```python
from build123d import *

# Parameters (mm, degrees)
SKETCH1_W              = 200
SKETCH1_H              = 60
BOSS_EXTRUDE1_DEPTH    = 12
M12_TAPPED_HOLE1_D     = 10.2
M12_TAPPED_HOLE1_DEPTH = 29.25
M12_TAPPED_HOLE1_TIP   = 3.064389157


with BuildPart() as part:
    # Sketch1 → Boss-Extrude1 (new body)
    with BuildSketch(Plane.XY):
        Rectangle(SKETCH1_W, SKETCH1_H)
    extrude(amount=BOSS_EXTRUDE1_DEPTH)

    # M12 Tapped Hole1
    with Locations(Plane.XY.offset(12)):
        with Locations((-80, 5), (80, 5)):
            Hole(M12_TAPPED_HOLE1_D / 2, depth=M12_TAPPED_HOLE1_DEPTH)
            with Locations((0, 0, -(M12_TAPPED_HOLE1_DEPTH + M12_TAPPED_HOLE1_TIP / 2))):  # 118° drill point
                Cone(0, M12_TAPPED_HOLE1_D / 2, M12_TAPPED_HOLE1_TIP, mode=Mode.SUBTRACT)


solid = part.part
```
Check sheet for the modelled part. Datum: model origin and axes. Units: mm. Give positions to 0.01 mm unless a question says otherwise; leave off trailing zeros. Write each loop counter-clockwise with the first axis right and the second up, starting at its lowest first coordinate (ties: lowest second). Pieces come first, ordered by that corner, then holes. Notation, with made-up numbers: (55.25, 68.25) -> (99.25, 68.25) arc R21 ccw to (99.25, 89.25) -> close; hole circle Ø3 at (2.25, 54). An arc over 180 degrees is marked (long way). Use CSV: the item, a comma, the result in double quotes. Start each with the question number.
Q1. Cross-section at B-B on y = 5. Enter the section's corners in (x, z), and give its area (3 significant figures).
Q2. Release check for a two-part mould opening along X. For faces 1 (the cylindrical face through (-74.905, 5.224, 5.916)), 2 (the flat face through (-1, -30, 6)), 3 (the flat face through (-100, 0, 6)) record: +X half, -X half, draft (parallel to the pull), parting line (faces both ways), or undercut.
Q3. Cross-section at A-A on x = -80. Enter the section's corners in (y, z).
Q4. Scan lines: line 1 along Y through (x, z) = (-80, 7); line 2 along X through (y, z) = (9, 7.5); line 3 along X through (y, z) = (6.5, 4). Record each from-to range of solid material in increasing order.
Q5. Depth check by flat-ended pin: P1, Ø10, axis at x = -68.5, y = 8.5, coming from the -Z side. Enter the tip coordinate at first touch or a pass-through.
Working result:
1,outline,"(-100, 0) -> (-85.1, 0) -> (-85.1, 12) -> (-100, 12) -> close; (-74.9, 0) -> (74.9, 0) -> (74.9, 12) -> (-74.9, 12) -> close; (85.1, 0) -> (100, 0) -> (100, 12) -> (85.1, 12) -> close"
1,area,"2,160 mm^2"
2,face 1,"undercut"
2,face 2,"draft"
2,face 3,"-X half"
3,outline,"(-30, 0) -> (-0.1, 0) -> (-0.1, 12) -> (-30, 12) -> close; (10.1, 0) -> (30, 0) -> (30, 12) -> (10.1, 12) -> close"
4,line 1,"y = -30 to -0.1, 10.1 to 30"
4,line 2,"x = -100 to -83.16, -76.84 to 76.84, 83.16 to 100"
4,line 3,"x = -100 to -84.87, -75.13 to 75.13, 84.87 to 100"
5,P1,"stops at z = 0"
